Check sheet for the modelled part. Datum: model origin and axes. Units: mm. Face numbers are marked on the shaded views. A direction names the side the tool comes from. Round coordinates to 2 decimals unless told otherwise and drop trailing zeros. Write each loop counter-clockwise with the first axis right and the second up, starting at its lowest first coordinate (ties: lowest second). Pieces come first, ordered by that corner, then holes. Notation, with made-up numbers: M 2,-19 L 10,-19 A22 ccw 10,10 Z; hole C 42,28 d4. An arc over 180 degrees is marked long. Answer in a Markdown table with one row per item.
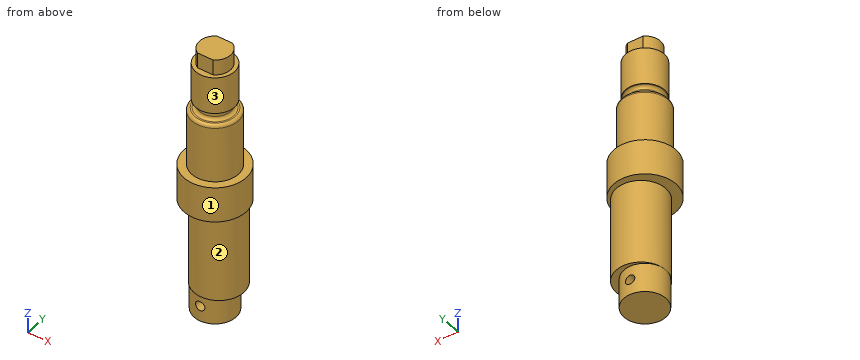
```python
from build123d import *

# Parameters (mm, degrees)
SKETCH2_R          = 13.5
EXTRUDE1_DEPTH     = 19
SKETCH3_R          = 16
EXTRUDE2_DEPTH     = 55
SKETCH4_R          = 20
EXTRUDE3_DEPTH     = 23
SKETCH5_R          = 15
EXTRUDE4_DEPTH     = 38
SKETCH6_R          = 10
EXTRUDE5_DEPTH     = 6
SKETCH7_R          = 12.5
EXTRUDE6_DEPTH     = 24
EXTRUDE7_DEPTH     = 10
SKETCH9_R          = 3
CUT_EXTRUDE1_DEPTH = 15
FILLET1_R          = 2


with BuildPart() as part:
    # Sketch2 → Extrude1 (new body)
    with BuildSketch(Plane.XY):
        Circle(SKETCH2_R)
    extrude(amount=EXTRUDE1_DEPTH)

    # Sketch3 → Extrude2 (add)
    with BuildSketch(Plane.XY.offset(19)):
        with Locations(Location((2.5, 0, 0), (0, 0, 179.999529266))):
            Circle(SKETCH3_R)
    extrude(amount=EXTRUDE2_DEPTH)

    # Sketch4 → Extrude3 (add)
    with BuildSketch(Plane.XY.offset(74)):
        Circle(SKETCH4_R)
    extrude(amount=EXTRUDE3_DEPTH)

    # Sketch5 → Extrude4 (add)
    with BuildSketch(Plane.XY.offset(97)):
        Circle(SKETCH5_R)
    extrude(amount=EXTRUDE4_DEPTH)

    # Sketch6 → Extrude5 (add)
    with BuildSketch(Plane.XY.offset(135)):
        Circle(SKETCH6_R)
    extrude(amount=EXTRUDE5_DEPTH)

    # Sketch7 → Extrude6 (add)
    with BuildSketch(Plane.XY.offset(141)):
        Circle(SKETCH7_R)
    extrude(amount=EXTRUDE6_DEPTH)

    # Sketch8 → Extrude7 (add)
    with BuildSketch(Plane.XY.offset(165)):
        with BuildLine():
            Line((-5, 8.660254038), (5, 8.660254038))
            ThreePointArc((5, 8.660254038), (10, 0), (5, -8.660254038))
            Line((5, -8.660254038), (-5, -8.660254038))
            ThreePointArc((-5, -8.660254038), (-10, 0), (-5, 8.660254038))
        make_face()
    extrude(amount=EXTRUDE7_DEPTH)

    # Sketch9 → Cut-Extrude1 (cut, symmetric)
    with BuildSketch(Plane(origin=(0, 0, 0), x_dir=(1, 0, 0), z_dir=(0, 1, 0))):
        with Locations(Location((0, -10, 0), (0, 0, 270))):
            Circle(SKETCH9_R)
    extrude(amount=CUT_EXTRUDE1_DEPTH, both=True, mode=Mode.SUBTRACT)

    # Fillet1
    fillet1_edges = [part.edges().sort_by_distance(p)[0] for p in [
        (-15, 0, 135),
        (-10, 0, 135),
        (-10, 0, 141),
    ]]
    fillet(fillet1_edges, radius=FILLET1_R)


solid = part.part
```
1. Go/stop test with flat-tipped pins: pin 1 (6 mm diameter, centred on y = -14, z = 98.5, fed in from -X); pin 2 (8 mm diameter, centred on y = -10, z = 52.5, fed in from +X); pin 3 (12 mm diameter, centred on x = 9, y = 14, fed in from +Z). Record where each tip stops, or that it passes through.
Found:
| item | result |
|---|---|
| pin 1 | stops at x = -16.43 |
| pin 2 | stops at x = 17.33 |
| pin 3 | stops at z = 165 |
2. Section check B-B, the plane z = 79. Record the cut outline in (x, y).
Found:
| item | result |
|---|---|
| outline | C 0,0 d40 |
3. Scan lines: L1, parallel to X at y = 0, z = 10; L2, parallel to Z at x = 0, y = -1.75; L3, parallel to Z at x = -14, y = -8. Record each from-to range of solid material in increasing order.
Found:
| item | result |
|---|---|
| L1 | x = -13.5 to -3, 3 to 13.5 |
| L2 | z = 0 to 7, 13 to 175 |
| L3 | z = 74 to 97 |
4. Access from +Z, -Z, +X, -X, +Y, -Y to the whole of each face (thin tool, end or side, straight path). Record for the marked faces 1, 2 and 3.
Found:
| item | result |
|---|---|
| face 1 | +Z, -Z |
| face 2 | -Z |
| face 3 | +Z |
5. Section check A-A, the plane z = 125. Record the cut outline in (x, y).
Found:
| item | result |
|---|---|
| outline | C 0,0 d30 |
